Geometry: final body of the model. Coordinates: model frame, mm. Round coordinates to 2 decimals unless told otherwise and drop trailing zeros. Write each loop counter-clockwise with the first axis right and the second up, starting at its lowest first coordinate (ties: lowest second). Pieces come first, ordered by that corner, then holes. Notation, with made-up numbers: (60.25, 88) - (83.25, 88) arc R9 ccw to (83.25, 94) - close; hole circle Ø4 at (1, 29). An arc over 180 degrees is marked (long way). Use a Markdown table: item, result. Add a question column.
```python
from build123d import *

# Parameters (mm, degrees)
SKETCH_1_W                   = 270
SKETCH_1_H                   = 192
EXTRUDE_1_DEPTH              = 6
SKETCH_2_W                   = 105
SKETCH_2_H                   = 32
CUT_EXTRUDE_1_DEPTH          = 12
HOLE_WIZARD_M8_1_D           = 6.8
HOLE_WIZARD_M8_1_DEPTH       = 19.75
HOLE_WIZARD_M8_1_TIP         = 2.042926105
HOLE_WIZARD_M4_1_D           = 3.3
CHAMFER_1_SIZE               = 5
FILLET_1_R                   = 10
HOLE_WIZARD_M8_2_D           = 6.8
HOLE_WIZARD_M8_3_D           = 9
HOLE_WIZARD_M8_3_DEPTH       = 24.5
HOLE_WIZARD_M8_3_CBORE_D     = 15
HOLE_WIZARD_M8_3_CBORE_DEPTH = 8.6
HOLE_WIZARD_M8_3_TIP         = 2.703872786
HOLE_WIZARD_M5_2_D           = 4.2
HOLE_WIZARD_M5_3_AT_2_COUNT  = 2
HOLE_WIZARD_M5_3_AT_2_PITCH  = 50


with BuildPart() as part:
    # 草图1 → 凸台-拉伸1 (new, symmetric)
    with BuildSketch(Plane.XY):
        Rectangle(SKETCH_1_W, SKETCH_1_H)
    extrude(amount=EXTRUDE_1_DEPTH, both=True)

    # 草图2 → 切除-拉伸1 (cut)
    with BuildSketch(Plane.XY.offset(6)):
        with Locations((-82.5, -80)):
            Rectangle(SKETCH_2_W, SKETCH_2_H)
        with Locations((82.5, -80)):
            Rectangle(SKETCH_2_W, SKETCH_2_H)
    extrude(amount=-CUT_EXTRUDE_1_DEPTH, mode=Mode.SUBTRACT)

    # M8 螺纹孔1
    with Locations(Plane.XY.offset(6)):
        with Locations((-45, 61), (45, 61)):
            Hole(HOLE_WIZARD_M8_1_D / 2, depth=HOLE_WIZARD_M8_1_DEPTH)
            with Locations((0, 0, -(HOLE_WIZARD_M8_1_DEPTH + HOLE_WIZARD_M8_1_TIP / 2))):  # 118° drill point
                Cone(0, HOLE_WIZARD_M8_1_D / 2, HOLE_WIZARD_M8_1_TIP, mode=Mode.SUBTRACT)

    # M4 螺纹孔1 (through all)
    with Locations(Plane.XY.offset(6)):
        with Locations((-7.5, -91.5), (7.5, -91.5), (-7.5, -51.5), (7.5, -51.5)):
            Hole(HOLE_WIZARD_M4_1_D / 2)

    # 倒角1
    chamfer_1_edges = [part.edges().sort_by_distance(p)[0] for p in [
        (-135, -64, 0),
        (-30, -96, 0),
        (30, -96, 0),
        (135, -64, 0),
        (-135, 96, 0),
        (135, 96, 0),
    ]]
    chamfer(chamfer_1_edges, length=CHAMFER_1_SIZE)

    # 圆角1
    fillet_1_edges = [part.edges().sort_by_distance(p)[0] for p in [
        (-30, -64, 0),
        (30, -64, 0),
    ]]
    fillet(fillet_1_edges, radius=FILLET_1_R)

    # Hole Wizard M8 _2 (through all)
    with Locations(Plane(origin=(0, 0, -6), x_dir=(-1, 0, 0), z_dir=(0, 0, -1))):
        with Locations((-45, -49), (45, -49), (-103, -42.5), (103, -42.5)):
            Hole(HOLE_WIZARD_M8_2_D / 2)

    # M8 六角凹头螺钉的柱形沉头孔3
    with Locations(Plane(origin=(0, 0, -6), x_dir=(-1, 0, 0), z_dir=(0, 0, -1))):
        with Locations((-50, 43.5), (-50, -6.5), (0, 43.5), (0, -6.5), (50, 43.5), (50, -6.5)):
            CounterBoreHole(HOLE_WIZARD_M8_3_D / 2, HOLE_WIZARD_M8_3_CBORE_D / 2, HOLE_WIZARD_M8_3_CBORE_DEPTH, depth=HOLE_WIZARD_M8_3_DEPTH)
            with Locations((0, 0, -(HOLE_WIZARD_M8_3_DEPTH + HOLE_WIZARD_M8_3_TIP / 2))):  # 118° drill point
                Cone(0, HOLE_WIZARD_M8_3_D / 2, HOLE_WIZARD_M8_3_TIP, mode=Mode.SUBTRACT)

    # M5 螺纹孔2 (through all)
    with Locations(Plane(origin=(0, 0, -6), x_dir=(-1, 0, 0), z_dir=(0, 0, -1))):
        with Locations((-7.5, 90), (7.5, 90)):
            Hole(HOLE_WIZARD_M5_2_D / 2)

    # 草图23 → M5 螺纹孔3 (revolve, cut)
    with BuildSketch(Plane(origin=(-135, -6.5, 0), x_dir=(0, 0, 1), z_dir=(0, 1, 0))):
        Polygon((0, 0), (0, 13.6618073), (2.1, 12.4), (2.1, 0), align=None)
    hole_wizard_m5_3 = revolve(axis=Axis((-141.35, -6.5, 0), (1, 0, 0)), mode=Mode.SUBTRACT)

    # M5 螺纹孔3 at 2: M5 螺纹孔3 ×2
    with Locations(*[(0, i * HOLE_WIZARD_M5_3_AT_2_PITCH, 0) for i in range(1, HOLE_WIZARD_M5_3_AT_2_COUNT)]):
        add(hole_wizard_m5_3, mode=Mode.SUBTRACT)

    # 镜向1: M5 螺纹孔3 across plane
    add(hole_wizard_m5_3.mirror(Plane(origin=(0, 0, 0), x_dir=(0, 0, 1), z_dir=(1, 0, 0))), mode=Mode.SUBTRACT)

    # 镜向1 copy 1 sketch → 镜向1 copy 1 (revolve, cut)
    with BuildSketch(Plane(origin=(135, 43.5, 0), x_dir=(0, 0, 1), z_dir=(0, 1, 0))):
        Polygon((0, 0), (0, -13.6618073), (2.1, -12.4), (2.1, 0), align=None)
    revolve(axis=Axis((141.35, 43.5, 0), (1, 0, 0)), mode=Mode.SUBTRACT)


solid = part.part
```
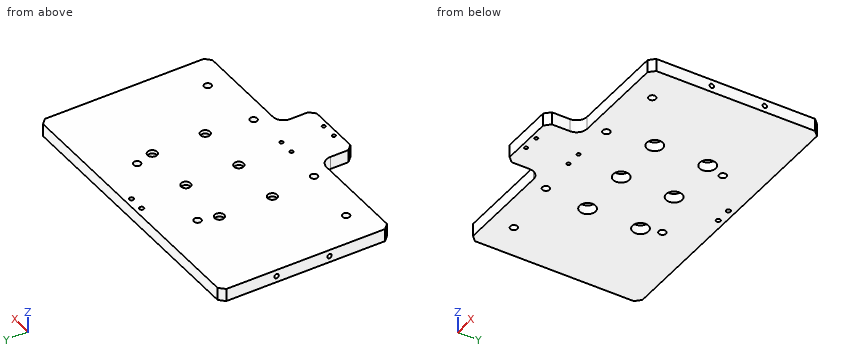
1) Section D-D, the plane x = -69.5. Return the cut outline in (y, z), then the cut area to 3 significant figures.
2) Section C-C, the plane x = 0. Return the cut outline in (y, z).
3) Section A-A, the plane x = 103. Return the cut outline in (y, z), then the cut area to 3 significant figures.
4) Pin query (flat end, axial travel): P1, Ø3.5, axis at x = -91.5, z = 2, coming from the -Y side; P2, Ø6, axis at y = -78.5, z = 0, coming from the -X side; P3, Ø4.5, axis at x = -3, y = 45, coming from the -Z side. Return the tip coordinate at first contact, or that it passes through.
5) Section B-B, the plane y = 61. Return the cut outline in (x, z).
6) Material intervals for L1, parallel to Y at x = 50, z = 4.25; L2, parallel to X at y = 50, z = -5; L3, parallel to Y at x = 103, z = -0.75, sorted ascending. Write a range as from..to.
Output values:
| question | item | result |
|---|---|---|
| 1 | outline | (-64, -6) - (96, -6) - (96, 6) - (-64, 6) - close |
| 1 | area | 1,920 mm^2 |
| 2 | outline | (-96, -6) - (-14, -6) - (-14, 2.6) - (-11, 2.6) - (-11, 6) - (-96, 6) - close; (-2, 2.6) - (1, 2.6) - (1, -6) - (36, -6) - (36, 2.6) - (39, 2.6) - (39, 6) - (-2, 6) - close; (48, 2.6) - (51, 2.6) - (51, -6) - (96, -6) - (96, 6) - (48, 6) - close |
| 3 | outline | (-64, -6) - (-45.9, -6) - (-45.9, 6) - (-64, 6) - close; (-39.1, -6) - (96, -6) - (96, 6) - (-39.1, 6) - close |
| 3 | area | 1,840 mm^2 |
| 4 | P1 | stops at y = -64 |
| 4 | P2 | stops at x = -30 |
| 4 | P3 | stops at z = 2.6 |
| 5 | outline | (-135, -6) - (-48.4, -6) - (-48.4, 6) - (-135, 6) - close; (-41.6, -6) - (41.6, -6) - (41.6, 6) - (-41.6, 6) - close; (48.4, -6) - (135, -6) - (135, 6) - (48.4, 6) - close |
| 6 | L1 | y = -64..-11, -2..39, 48..96 |
| 6 | L2 | x = -135..-53.74, -46.26..-3.74, 3.74..46.26, 53.74..135 |
| 6 | L3 | y = -64..-45.9, -39.1..96 |
